```python
from build123d import *

# Parameters (mm, degrees)
SKETCH_1_W               = 12
SKETCH_1_H               = 12
SKETCH_1_W_2             = 10
SKETCH_1_H_2             = 10
EXTRUDE_1_DEPTH          = 516
CUT_EXTRUDE_1_DEPTH      = 517.174389136
CUT_EXTRUDE_1_DEPTH_BACK = 517.174389136
SKETCH_2_R               = 1.55
SKETCH_3_W               = 12
SKETCH_3_H               = 12
SKETCH_3_W_2             = 10
SKETCH_3_H_2             = 10
CUT_EXTRUDE_2_DEPTH      = 8


with BuildPart() as part:
    # 草图1 → 凸台-拉伸1 (new body)
    with BuildSketch(Plane.XY):
        Rectangle(SKETCH_1_W, SKETCH_1_H)
        Rectangle(SKETCH_1_W_2, SKETCH_1_H_2, mode=Mode.SUBTRACT)
    extrude(amount=EXTRUDE_1_DEPTH)

    # 草图2 → 切除-拉伸1 (cut, two sides: drawn at the far end of the back side and taken through both)
    with BuildSketch(Plane.ZY.offset(6).offset(-CUT_EXTRUDE_1_DEPTH_BACK)):
        with Locations(Location((50, 0, 0), (0, 0, 180))):
            Circle(SKETCH_2_R)
        with Locations(Location((468.132973417, 0, 0), (0, 0, 180))):
            Circle(SKETCH_2_R)
        with Locations(Location((503.132973417, 0, 0), (0, 0, 180))):
            Circle(SKETCH_2_R)
    extrude(amount=CUT_EXTRUDE_1_DEPTH + CUT_EXTRUDE_1_DEPTH_BACK, mode=Mode.SUBTRACT)

    # 草图3 → 切除-拉伸2 (cut)
    with BuildSketch(Plane.XY.offset(516)):
        Rectangle(SKETCH_3_W, SKETCH_3_H)
        Rectangle(SKETCH_3_W_2, SKETCH_3_H_2, mode=Mode.SUBTRACT)
    extrude(amount=-CUT_EXTRUDE_2_DEPTH, mode=Mode.SUBTRACT)


solid = part.part
```
Check sheet for the modelled part. Datum: model origin and axes. Units: mm. A direction names the side the tool comes from. Coordinates: 2 decimals unless noted, no trailing zeros. Loops run counter-clockwise (first coordinate to the right, second up) from the corner with the lowest first, then second, coordinate; pieces in that order, holes last. Notation, with made-up numbers: M 46.5,-19 L 98.5,-19 A13 cw 98.5,-8 Z; hole C -23,3 d10. An arc over 180 degrees is marked long. Answer as a JSON object with one key per item and string values.
1. Release check for a two-part mould opening along Y. For faces 3 (the flat face through (6, 0, 250)), 4 (the flat face through (-5, 0, 250)), 5 (the flat face through (0, -6, 250)) record: pulls with the +Y half, pulls with the -Y half, needs draft (parallel to the pull), parting line crosses it, or undercut.
Outcome:
{"face 3": "needs draft", "face 4": "undercut", "face 5": "pulls with the -Y half"}
2. Scan lines: L1, parallel to Y at x = 1.5, z = 307; L2, parallel to Y at x = 5.3, z = 50. Record each from-to range of solid material in increasing order. Write a range as from..to.
Outcome:
{"L1": "-6..-5, 5..6", "L2": "-6..-1.55, 1.55..6"}
3. Sectioned sample at B-B on z = 256. Record the cut outline in (x, y), and give its area (3 significant figures).
Outcome:
{"outline": "M -6,-6 L 6,-6 L 6,6 L -6,6 Z; hole M -5,-5 L 5,-5 L 5,5 L -5,5 Z", "area": "44.0 mm²"}
4. Sectioned sample at A-A on x = -2.5. Record the cut outline in (y, z), and give its area (3 significant figures).
Outcome:
{"outline": "M -6,0 L -5,0 L -5,508 L -6,508 Z; M 5,0 L 6,0 L 6,508 L 5,508 Z", "area": "1,020 mm²"}
5. Access from +Z, -Z, +X, -X, +Y, -Y to the whole of each face (thin tool, end or side, straight path). Record for faces 1 (the flat face through (5, 0, 250)), 2 (the flat face through (5.2, 0.1, 508)).
Outcome:
{"face 1": "+Z, -Z", "face 2": "+Z, +X, -X, +Y, -Y"}
